Input: dimensioned drawing with shaded views. Units: mm. Origin: part minimum x, y, z. Give positions to 0.01 mm unless a question says otherwise; leave off trailing zeros. Write each loop counter-clockwise with the first axis right and the second up, starting at its lowest first coordinate (ties: lowest second). Pieces come first, ordered by that corner, then holes.
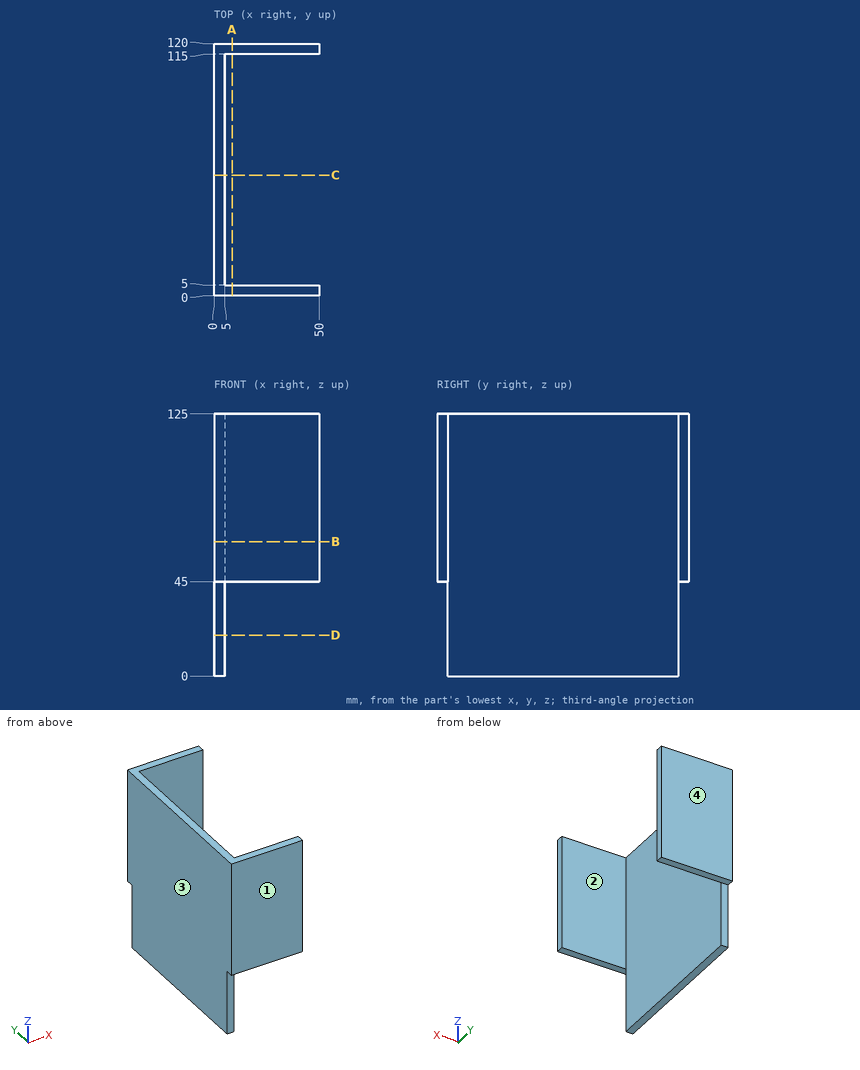
Item 1: Section D-D, the plane z = 19.5. Return the cut outline in (x, y), plus the area to 3 significant figures.
Found:
outline: (0, 5) - (5, 5) - (5, 115) - (0, 115) - close
area: 550 mm2
Item 2: Line query: L1, parallel to Y at x = 25, z = 118; L2, parallel to X at y = 103, z = 63. Output: solid intervals per line, ascending.
Found:
L1: y = 0 to 5, 115 to 120
L2: x = 0 to 5
Item 3: Section C-C, the plane y = 57.5. Return the cut outline in (x, z).
Found:
outline: (0, 0) - (5, 0) - (5, 125) - (0, 125) - close
Item 4: Section A-A, the plane x = 8.5. Return the cut outline in (y, z).
Found:
outline: (0, 45) - (5, 45) - (5, 125) - (0, 125) - close; (115, 45) - (120, 45) - (120, 125) - (115, 125) - close
Item 5: Pull-direction query (Y, two-part tool) for the marked faces 1, 2, 3 and 4; classes: +Y half, -Y half, draft (parallel to the pull), parting line (faces both ways), or undercut.
Found:
face 1: -Y half
face 2: undercut
face 3: draft
face 4: +Y half
Item 6: Pin query (flat end, axial travel): pin 1 Ø5.5 at (x, z) = (3.5, 13) entering from -Y; pin 2 Ø12 at (x, y) = (17, 107.5) entering from -Z; pin 3 Ø2.5 at (x, y) = (22.5, 1.5) entering from -Z; pin 4 Ø3 at (y, z) = (30.5, 98.5) entering from +X. Return the tip coordinate at first contact, or that it passes through.
Found:
pin 1: stops at y = 5
pin 2: passes through
pin 3: stops at z = 45
pin 4: stops at x = 5
Item 7: Section B-B, the plane z = 64. Return the cut outline in (x, y).
Found:
outline: (0, 0) - (50, 0) - (50, 5) - (5, 5) - (5, 115) - (50, 115) - (50, 120) - (0, 120) - close
